Source: CAD feature listing. Evaluate the final solid. Frame: model axes, mm. A direction names the side the tool comes from. Give positions to 0.01 mm unless a question says otherwise; leave off trailing zeros. Write each loop counter-clockwise with the first axis right and the second up, starting at its lowest first coordinate (ties: lowest second). Pieces come first, ordered by that corner, then holes. Notation, with made-up numbers: M -12,19.5 L 40,19.5 A36 cw 40,53.5 Z; hole C -11.5,59.5 d11. An arc over 180 degrees is marked long. Return JSON: item names as keys, results as strings.
```python
from build123d import *


with BuildPart() as part:
    # Sketch1 → Revolve1 (revolve)
    with BuildSketch(Plane.XZ.offset(-889.976481234), mode=Mode.PRIVATE) as revolve1_sk:
        Polygon((533.730642584, -100.892981355), (521.230642584, -100.892981355), (521.230642584, -390.892981355), (533.730642584, -390.892981355), (533.730642584, -300.892981355), (535.230642584, -300.892981355), (535.230642584, -240.892981355), (533.730642584, -240.892981355), align=None)
    revolve(revolve1_sk.sketch.rotate(Axis((521.230642584, 889.976481234, -100.892981355), (0, 0, -1)), 180), axis=Axis((521.230642584, 889.976481234, -100.892981355), (0, 0, -1)))


solid = part.part
```
1) Cut plane A-A, the plane y = 880.25. Return the cut outline in (x, z), then the cut area to 3 significant figures.
Numbers:
{"outline": "M 511.16,-300.89 L 513.38,-300.89 L 513.38,-390.89 L 529.08,-390.89 L 529.08,-300.89 L 531.3,-300.89 L 531.3,-240.89 L 529.08,-240.89 L 529.08,-100.89 L 513.38,-100.89 L 513.38,-240.89 L 511.16,-240.89 Z", "area": "4,820 mm²"}
2) Set-up query: faces 1 (the face through (507.877, 894.182, -270.473)), 2 (the face through (523.94, 877.774, -169.913)), 3 (the face through (523.94, 877.774, -345.263)). Return all of +Z, -Z, +X, -X, +Y, -Y with unobstructed straight access to the full face (end or side cutting, diameter ignored); none if empty.
Numbers:
{"face 1": "+Z, -Z", "face 2": "+Z", "face 3": "-Z"}
3) Cut plane B-B, the plane x = 527.25. Return the cut outline in (y, z).
Numbers:
{"outline": "M 877.34,-300.89 L 879.02,-300.89 L 879.02,-390.89 L 900.93,-390.89 L 900.93,-300.89 L 902.62,-300.89 L 902.62,-240.89 L 900.93,-240.89 L 900.93,-100.89 L 879.02,-100.89 L 879.02,-240.89 L 877.34,-240.89 Z"}
4) Cut plane D-D, the plane z = -175.5. Return the cut outline in (x, y), then the cut area to 3 significant figures.
Numbers:
{"outline": "C 521.23,889.98 d25", "area": "491 mm²"}
5) Line query: line 1 (X direction, y = 889.75, z = -226.5); line 2 (Z direction, x = 510, y = 898.25); line 3 (X direction, y = 897.5, z = -228). Output: solid intervals per line, ascending. Write a range as [from, to].
Numbers:
{"line 1": "x = [508.73, 533.73]", "line 2": "z = [-300.89, -240.89]", "line 3": "x = [511.25, 531.21]"}
6) Cut plane C-C, the plane z = -280. Return the cut outline in (x, y).
Numbers:
{"outline": "C 521.23,889.98 d28"}
7) Contact query for flat-ended pins moving along their axis: pin 1 Ø1.5 at (y, z) = (886, -130.5) entering from -X; pin 2 Ø12 at (x, z) = (532, -144.5) entering from -Y; pin 3 Ø12 at (x, z) = (527, -276) entering from +Y; pin 4 Ø2 at (y, z) = (896.5, -172) entering from +X. Output: stop coordinate, or through.
Numbers:
{"pin 1": "stops at x = 509.15", "pin 2": "stops at y = 878.42", "pin 3": "stops at y = 903.98", "pin 4": "stops at x = 532.44"}
